Verification items for the finished model (mm, model axes). Round coordinates to 2 decimals unless told otherwise and drop trailing zeros. Write each loop counter-clockwise with the first axis right and the second up, starting at its lowest first coordinate (ties: lowest second). Pieces come first, ordered by that corner, then holes. Notation, with made-up numbers: M 53.25,70 L 109.25,70 A24 ccw 109.25,108 Z; hole C -20.75,22.5 d8. An arc over 180 degrees is marked long. Answer in a Markdown table with one row per item. Add a question column.
1. Draft check along Y on faces 1 (the flat face through (0, 0, 4.2)), 2 (the flat face through (1.014, 1.724, -43.521)), 3 (the conical face through (0.474, 2.133, 2.433)). Enter one of: pulls with the +Y half, pulls with the -Y half, needs draft (parallel to the pull), parting line crosses it, or undercut.
2. Sectioned sample at A-A on z = -20. Record the cut outline in (x, y).
3. Go/stop test with flat-tipped pins: pin 1 Ø2 at (x, y) = (-4.5, -3) entering from -Z; pin 2 Ø5 at (y, z) = (3.5, -9.5) entering from -X; pin 3 Ø1 at (x, z) = (4, -30.5) entering from -Y; pin 4 Ø3 at (x, y) = (-3, 0.5) entering from -Z. Record where each tip stops, or that it passes through.
4. Material ranges on probe 1 along X at (y, z) = (-0.25, -51); probe 2 along Y at (x, z) = (0, -46.5); probe 3 along Z at (x, y) = (-0.25, 4), recorded low to high.
```python
from build123d import *

# Parameters (mm, degrees)
CUT_EXTRUDE1_DEPTH = 5
SKETCH5_W          = 12
SKETCH5_H          = 4
CUT_EXTRUDE2_DEPTH = 3


with BuildPart() as part:
    # Sketch1 → Revolve1 (revolve)
    with BuildSketch(Plane(origin=(0, 0, 0), x_dir=(0, 0, -1), z_dir=(1, 0, 0)), mode=Mode.PRIVATE) as revolve1_sk:
        Polygon((0, 0), (0, 5.3), (0.7, 6), (53.3, 6), (54, 5.3), (54, 0), align=None)
    revolve(revolve1_sk.sketch.rotate(Axis((0, 0, -54), (0, 0, 1)), 270), axis=Axis((0, 0, -54), (0, 0, 1)))

    # Sketch2 → Cut-Revolve1 (revolve, cut)
    with BuildSketch(Plane(origin=(0, 0, 0), x_dir=(0, 0, -1), z_dir=(1, 0, 0)), mode=Mode.PRIVATE) as cut_revolve1_sk:
        Polygon((37, 0), (37, 3.4585), (49, 3.4585), (49, 4), (53.2, 4), (54, 4.8), (54, 0), align=None)
    revolve(cut_revolve1_sk.sketch.rotate(Axis((0, 0, -54), (0, 0, 1)), 270), axis=Axis((0, 0, -54), (0, 0, 1)), mode=Mode.SUBTRACT)

    # Sketch3 → Revolve2 (revolve)
    with BuildSketch(Plane(origin=(0, 0, 0), x_dir=(0, 0, -1), z_dir=(1, 0, 0)), mode=Mode.PRIVATE) as revolve2_sk:
        with BuildLine():
            Line((-4.2, 0), (-4.2, 1.762627227))
            ThreePointArc((-4.2, 1.762627227), (-4.150941916, 1.893839033), (-4.02783462, 1.960680841))
            Line((-4.02783462, 1.960680841), (2.3, 2.85))
            Line((2.3, 2.85), (2.3, 0))
            Line((2.3, 0), (-4.2, 0))
        make_face()
    revolve(revolve2_sk.sketch.rotate(Axis((0, 0, -2.3), (0, 0, 1)), 90), axis=Axis((0, 0, -2.3), (0, 0, 1)))

    # Sketch4 → Cut-Extrude1 (cut)
    with BuildSketch(Plane.XY.offset(-54)):
        Polygon((-4, -2.309401077), (0, -4.618802154), (4, -2.309401077), (4, 2.309401077), (0, 4.618802154), (-4, 2.309401077), align=None)
    extrude(amount=CUT_EXTRUDE1_DEPTH, mode=Mode.SUBTRACT)

    # Sketch5 → Revolve3 (revolve)
    with BuildSketch(Plane(origin=(0, 0, 0), x_dir=(0, 0, -1), z_dir=(1, 0, 0)), mode=Mode.PRIVATE) as revolve3_sk:
        with Locations((39, 2)):
            Rectangle(SKETCH5_W, SKETCH5_H)
    revolve(revolve3_sk.sketch.rotate(Axis((0, 0, -45), (0, 0, 1)), 270), axis=Axis((0, 0, -45), (0, 0, 1)))

    # Sketch6 → Cut-Extrude2 (cut)
    with BuildSketch(Plane.XY.offset(-45)):
        Polygon((-2, -1.154700538), (0, -2.309401077), (2, -1.154700538), (2, 1.154700538), (0, 2.309401077), (-2, 1.154700538), align=None)
    extrude(amount=CUT_EXTRUDE2_DEPTH, mode=Mode.SUBTRACT)

    # Sketch7 → Cut-Revolve2 (revolve, cut)
    with BuildSketch(Plane(origin=(0, 0, 0), x_dir=(0, 0, -1), z_dir=(1, 0, 0)), mode=Mode.PRIVATE) as cut_revolve2_sk:
        Polygon((40.845299462, 0), (42, 2), (42, 0), align=None)
    revolve(cut_revolve2_sk.sketch.rotate(Axis((0, 0, -42), (0, 0, 1)), 120.000000088), axis=Axis((0, 0, -42), (0, 0, 1)), mode=Mode.SUBTRACT)


solid = part.part
```
Geometry check:
| question | item | result |
|---|---|---|
| 1 | face 1 | needs draft |
| 1 | face 2 | undercut |
| 1 | face 3 | parting line crosses it |
| 2 | outline | C 0,0 d12 |
| 3 | pin 1 | stops at z = -54 |
| 3 | pin 2 | stops at x = -5.92 |
| 3 | pin 3 | stops at y = -4.87 |
| 3 | pin 4 | stops at z = -53.74 |
| 4 | probe 1 | x = -5.99 to -4, 4 to 5.99 |
| 4 | probe 2 | y = -6 to -3.46, 3.46 to 6 |
| 4 | probe 3 | z = -49 to 0 |
